Input: part model. Units: mm. Frame: model coordinates. A direction names the side the tool comes from. Coordinates: 2 decimals unless noted, no trailing zeros. Loops run counter-clockwise (first coordinate to the right, second up) from the corner with the lowest first, then second, coordinate; pieces in that order, holes last.
```python
from build123d import *

# Parameters (mm, degrees)
SKETCH_1_R                  = 52
EXTRUDE_1_DEPTH             = 55
SKETCH_2_R                  = 70
EXTRUDE_2_DEPTH             = 10
EXTRUDE_START               = 110
EXTRUDE_3_DEPTH             = 110
EXTRUDE_4_REACH             = 120.427
EXTRUDE_4_DIRECTION_2_REACH = 120.427
SKETCH_5_R                  = 4
CUT_EXTRUDE_1_DEPTH         = 229
SKETCH_6_R                  = 3.3
CUT_EXTRUDE_2_DEPTH         = 68
CUT_EXTRUDE_START           = -30
SKETCH_8_R                  = 8
CUT_EXTRUDE_4_DEPTH         = 168
CHAMFER_1_SIZE              = 2


with BuildPart() as part:
    # 草图1 → 凸台-拉伸1 (new, symmetric)
    with BuildSketch(Plane.XY):
        Circle(SKETCH_1_R)
    extrude(amount=EXTRUDE_1_DEPTH, both=True)

    # 草图2 → 凸台-拉伸2 (add)
    with BuildSketch(Plane.XY.offset(55)):
        Circle(SKETCH_2_R)
    extrude(amount=EXTRUDE_2_DEPTH)

    # 镜向1: part across plane


with BuildPart() as part_1:
    add(part.part)
    add(part.part.mirror(Plane.XY))

    # 草图3 → 凸台-拉伸3 (add)
    with BuildSketch(Plane.XY.offset(-55).offset(EXTRUDE_START)):
        with BuildLine():
            ThreePointArc((67.61480784, 18.117333157), (-18.117333157, 67.61480784), (-67.61480784, -18.117333157))
            Line((-67.61480784, -18.117333157), (-50.228142967, -13.458590345))
            ThreePointArc((-50.228142967, -13.458590345), (-13.458590345, 50.228142967), (50.228142967, 13.458590345))
            Line((50.228142967, 13.458590345), (67.61480784, 18.117333157))
        make_face()
    extrude(amount=-EXTRUDE_3_DEPTH)

    # 凸台-拉伸4: up to this face of the body (flat: up to its plane)
    extrude_4_end = Plane(part_1.part.faces().sort_by_distance((0, 0, 65))[0])
    # 草图4 → 凸台-拉伸4 (add, up to the picked face)
    with BuildSketch(Plane.XY, mode=Mode.PRIVATE) as extrude_4_sk1:
        with BuildLine():
            Line((23.122839281, 70), (0, 70))
            ThreePointArc((0, 70), (42.613300031, 55.53473382), (67.61480784, 18.117333157))
            Line((67.61480784, 18.117333157), (150, 55))
            Line((150, 55), (200, 55))
            Line((200, 55), (200, 70))
            Line((200, 70), (158.152049004, 70))
            Line((158.152049004, 70), (23.122839281, 70))
        make_face()
    extrude_4_tool1 = split(extrude(extrude_4_sk1.sketch, amount=EXTRUDE_4_REACH, mode=Mode.PRIVATE), bisect_by=extrude_4_end, keep=Keep.BOTH, mode=Mode.PRIVATE)
    # 草图4 → 凸台-拉伸4 (add, up to the picked face)
    with BuildSketch(Plane.XY, mode=Mode.PRIVATE) as extrude_4_sk2:
        Polygon((33.122839281, 80), (23.122839281, 70), (158.152049004, 70), (148.152049004, 80), align=None)
    extrude_4_tool2 = split(extrude(extrude_4_sk2.sketch, amount=EXTRUDE_4_REACH, mode=Mode.PRIVATE), bisect_by=extrude_4_end, keep=Keep.BOTH, mode=Mode.PRIVATE)
    add(extrude_4_tool1.solids().sort_by(Axis((103.613169, 54.432495, 0), (0, 0, 1)))[0])
    add(extrude_4_tool2.solids().sort_by(Axis((90.637444, 74.866698, 0), (0, 0, 1)))[0])

    # 凸台-拉伸4 direction 2: up to this face of the body (flat: up to its plane)
    extrude_4_direction_2_end = Plane(part_1.part.faces().sort_by_distance((0, 0, -65))[0])
    # 草图4 → 凸台-拉伸4 direction 2 (add, up to the picked face)
    with BuildSketch(Plane.XY, mode=Mode.PRIVATE) as extrude_4_direction_2_sk1:
        with BuildLine():
            Line((23.122839281, 70), (0, 70))
            ThreePointArc((0, 70), (42.613300031, 55.53473382), (67.61480784, 18.117333157))
            Line((67.61480784, 18.117333157), (150, 55))
            Line((150, 55), (200, 55))
            Line((200, 55), (200, 70))
            Line((200, 70), (158.152049004, 70))
            Line((158.152049004, 70), (23.122839281, 70))
        make_face()
    extrude_4_direction_2_tool1 = split(extrude(extrude_4_direction_2_sk1.sketch, amount=-EXTRUDE_4_DIRECTION_2_REACH, mode=Mode.PRIVATE), bisect_by=extrude_4_direction_2_end, keep=Keep.BOTH, mode=Mode.PRIVATE)
    # 草图4 → 凸台-拉伸4 direction 2 (add, up to the picked face)
    with BuildSketch(Plane.XY, mode=Mode.PRIVATE) as extrude_4_direction_2_sk2:
        Polygon((33.122839281, 80), (23.122839281, 70), (158.152049004, 70), (148.152049004, 80), align=None)
    extrude_4_direction_2_tool2 = split(extrude(extrude_4_direction_2_sk2.sketch, amount=-EXTRUDE_4_DIRECTION_2_REACH, mode=Mode.PRIVATE), bisect_by=extrude_4_direction_2_end, keep=Keep.BOTH, mode=Mode.PRIVATE)
    add(extrude_4_direction_2_tool1.solids().sort_by(Axis((103.613169, 54.432495, 0), (0, 0, -1)))[0])
    add(extrude_4_direction_2_tool2.solids().sort_by(Axis((90.637444, 74.866698, 0), (0, 0, -1)))[0])

    # 草图5 → 切除-拉伸1 (cut)
    with BuildSketch(Plane.XY.offset(65)):
        with Locations(Location((-43.16038802, -41.679502228, 0), (0, 0, 180))):
            Circle(SKETCH_5_R)
        with Locations(Location((14.515313736, -58.217743577, 0), (0, 0, 180))):
            Circle(SKETCH_5_R)
    extrude(amount=-CUT_EXTRUDE_1_DEPTH, mode=Mode.SUBTRACT)

    # 草图6 → 切除-拉伸2 (cut)
    with BuildSketch(Plane(origin=(0, 80, 0), x_dir=(1, 0, 0), z_dir=(0, 1, 0))):
        with Locations(Location((130, 50, 0), (0, 0, 270))):
            Circle(SKETCH_6_R)
        with Locations(Location((130, -50, 0), (0, 0, 270))):
            Circle(SKETCH_6_R)
    extrude(amount=-CUT_EXTRUDE_2_DEPTH, mode=Mode.SUBTRACT)

    # 草图8 → 切除-拉伸4 (cut)
    with BuildSketch(Plane(origin=(0, 80, 0), x_dir=(1, 0, 0), z_dir=(0, 1, 0)).offset(CUT_EXTRUDE_START)):
        with Locations(Location((130, 50, 0), (0, 0, 270))):
            Circle(SKETCH_8_R)
        with Locations(Location((130, -50, 0), (0, 0, 270))):
            Circle(SKETCH_8_R)
    extrude(amount=-CUT_EXTRUDE_4_DEPTH, mode=Mode.SUBTRACT)

    # 倒角1
    chamfer_1_edges = [part_1.edges().sort_by_distance(p)[0] for p in [
        (-42.613300031, -55.53473382, -65),
        (-42.613300031, -55.53473382, 65),
        (11.561419641, 70, 65),
        (28.122839281, 75, 65),
        (90.637444143, 80, 65),
        (153.152049004, 75, 65),
        (179.076024502, 70, 65),
        (200, 70, 0),
        (200, 62.5, 65),
        (200, 55, 0),
        (175, 55, 65),
        (108.80740392, 36.558666579, 65),
        (108.80740392, 36.558666579, -65),
        (11.561419641, 70, -65),
        (28.122839281, 75, -65),
        (90.637444143, 80, -65),
        (200, 62.5, -65),
        (175, 55, -65),
    ]]
    chamfer(chamfer_1_edges, length=CHAMFER_1_SIZE)


solid = part_1.part
```
Item 1: Section query D-D (x = 103.5). Output: boundary loops of the cut face in (y, z).
Result:
outline: (34.18, -63) - (36.37, -65) - (78, -65) - (80, -63) - (80, 63) - (78, 65) - (36.37, 65) - (34.18, 63) - close
Item 2: Section query B-B (z = 50). Output: boundary loops of the cut face in (x, y), then the cut area to 3 significant figures.
Result:
outline: (-67.61, -18.12) - (-50.23, -13.46) arc R52 ccw to (50.23, 13.46) - (67.61, 18.12) - (122, 42.46) - (122, 50) - (126.7, 50) - (126.7, 80) - (33.12, 80) - (23.12, 70) - (0, 70) arc R70 ccw to start; (133.3, 50) - (138, 50) - (138, 49.63) - (150, 55) - (198, 55) - (200, 57) - (200, 68) - (198, 70) - (158.15, 70) - (148.15, 80) - (133.3, 80) - close
area: 17,300 mm2
Item 3: Mould query, pull axis X, two halves, no side actions, for faces 1 (the face through (15.382, -54.313, -59.93)), 2 (the face through (12, 70, 1)), 3 (the face through (108.23, 36.3, 0.88)), 4 (the face through (28.621, 74.064, -64.014)). Classes: +X half, -X half, draft (parallel to the pull), parting line (faces both ways), or undercut.
Result:
face 1: undercut
face 2: draft
face 3: +X half
face 4: -X half
Item 4: Contact query for flat-ended pins moving along their axis: P1, Ø10, axis at x = 59.5, z = -15.5, coming from the -Y side; P2, Ø10, axis at y = 9.5, z = 6.5, coming from the -X side; P3, Ø17.5, axis at x = 129, z = 50.5, coming from the -Y side. Output: stop coordinate, or through.
Result:
P1: stops at y = 14.6
P2: stops at x = -69.86
P3: stops at y = 41.68
Item 5: Line query: L1, parallel to Z at x = 130, y = 60; L2, parallel to Z at x = 130, y = 48; L3, parallel to Y at x = 189, z = -39.5. Output: solid intervals per line, ascending.
Result:
L1: z = -65 to -53.3, -46.7 to 46.7, 53.3 to 65
L2: z = -64.78 to -58, -42 to 42, 58 to 64.78
L3: y = 55 to 70
Item 6: Section query C-C (z = -13.5). Output: boundary loops of the cut face in (x, y), then the cut area to 3 significant figures.
Result:
outline: (-67.61, -18.12) - (-50.23, -13.46) arc R52 ccw to (50.23, 13.46) - (67.61, 18.12) - (150, 55) - (198, 55) - (200, 57) - (200, 68) - (198, 70) - (158.15, 70) - (148.15, 80) - (33.12, 80) - (23.12, 70) - (0, 70) arc R70 ccw to start
area: 17,600 mm2
Item 7: Section query A-A (y = 0). Output: boundary loops of the cut face in (x, z), then the cut area to 3 significant figures.
Result:
outline: (-70, -63) - (-68, -65) - (68, -65) - (70, -63) - (70, -55) - (52, -55) - (52, 55) - (70, 55) - (70, 63) - (68, 65) - (-68, 65) - (-70, 63) - close
area: 16,200 mm2
Item 8: Reachability of faces 5 (the face through (200, 62, 1)), 6 (the face through (122.19, 47.12, -51.73)) from +Z, -Z, +X, -X, +Y, -Y: full face, straight path, thin tool, end or side. Return the list, or none.
Result:
face 5: +Z, -Z, +X, +Y, -Y
face 6: -Y
